Source: CAD feature listing. Evaluate the final solid. Frame: model axes, mm. A direction names the side the tool comes from. Give positions to 0.01 mm unless a question says otherwise; leave off trailing zeros. Loops run counter-clockwise (first coordinate to the right, second up) from the corner with the lowest first, then second, coordinate; pieces in that order, holes last. Notation, with made-up numbers: (29.25, 37) -> (38.25, 37) arc R18 ccw to (38.25, 54) -> close; hole circle Ø2 at (32.5, -11.5). An arc over 180 degrees is marked (long way). Return JSON: item names as keys, results as strings. Group by question number.
(1) Cut plane C-C on y = 28. Return loops of the section in (x, z).
(2) Access query for faces 4 (the face through (-35, 20, -22.5)), 5 (the face through (-1, 47, 32)), 6 (the face through (35, 20, -22.5)). Directions: +Z, -Z, +X, -X, +Y, -Y. A direction counts if a zero-diameter tool reaches every point of the face in a straight line with its end or side. Return the directions, or none.
(3) Ray query, line 1 (Z direction, x = 32.5, y = 18.5); line 2 (Y direction, x = -35.5, z = 12.5); line 3 (Z direction, x = 6.5, y = 15). Return the intervals inside material, ascending. Write a range as from..to.
(4) Cut plane D-D on x = -31.5. Return loops of the section in (y, z).
(5) Cut plane B-B on x = 0. Return loops of the section in (y, z).
(6) Cut plane A-A on z = 0. Return loops of the section in (x, y).
(7) Pin query (flat end, axial travel): pin 1 (6.5 mm diameter, centred on x = -7.5, y = 45.5, fed in from +Z); pin 2 (3 mm diameter, centred on x = 14, y = 47, fed in from -Z); pin 3 (6.5 mm diameter, centred on x = -5.5, z = -35.5, fed in from +Y); pin 4 (10 mm diameter, centred on y = 29, z = 0.5, fed in from +X). Return the tip coordinate at first contact, or that it passes through.
(8) Draft query along Z for faces 1 (the face through (37, 40, 0)), 2 (the face through (-1, 22, 38)), 3 (the face through (-1, 44, 35)). Return one class per face: released by +Z, released by -Z, zero draft, split by the parting line, or undercut.
```python
from build123d import *

# Parameters (mm, degrees)
CHANNEL_BODY_DEPTH      = 40
TOP_PLATE_SKETCH_W      = 100
TOP_PLATE_SKETCH_H      = 76
TOP_PLATE_DEPTH         = 10
BORE_SKETCH_R           = 12.5
BORE_25_DEPTH           = 56
GUIDE_GROOVES_SKETCH_W  = 100
GUIDE_GROOVES_SKETCH_H  = 6
GUIDE_GROOVES_6X6_DEPTH = 6


with BuildPart() as part:
    # Channel Profile Sketch → Channel Body (new body)
    with BuildSketch(Plane(origin=(0, 0, 0), x_dir=(1, 0, 0), z_dir=(0, 1, 0))):
        with BuildLine():
            Line((-50, 22.5), (-20.093531297, 22.5))
            ThreePointArc((-20.093531297, 22.5), (-17.330574806, 20.668790584), (-17.940652944, 17.410714286))
            ThreePointArc((-17.940652944, 17.410714286), (-25, 0), (-17.940652944, -17.410714286))
            ThreePointArc((-17.940652944, -17.410714286), (-17.330574806, -20.668790584), (-20.093531297, -22.5))
            Line((-20.093531297, -22.5), (-50, -22.5))
            Line((-50, -22.5), (-50, -38))
            Line((-50, -38), (50, -38))
            Line((50, -38), (50, -22.5))
            Line((50, -22.5), (20.093531297, -22.5))
            ThreePointArc((20.093531297, -22.5), (17.330574806, -20.668790584), (17.940652944, -17.410714286))
            ThreePointArc((17.940652944, -17.410714286), (25, 0), (17.940652944, 17.410714286))
            ThreePointArc((17.940652944, 17.410714286), (17.330574806, 20.668790584), (20.093531297, 22.5))
            Line((20.093531297, 22.5), (50, 22.5))
            Line((50, 22.5), (50, 38))
            Line((50, 38), (-50, 38))
            Line((-50, 38), (-50, 22.5))
        make_face()
    extrude(amount=CHANNEL_BODY_DEPTH)

    # Top Plate Sketch → Top Plate (add)
    with BuildSketch(Plane(origin=(0, 40, 0), x_dir=(1, 0, 0), z_dir=(0, 1, 0))):
        Rectangle(TOP_PLATE_SKETCH_W, TOP_PLATE_SKETCH_H)
    extrude(amount=TOP_PLATE_DEPTH)

    # Bore Sketch → Bore Ø25 (cut)
    with BuildSketch(Plane(origin=(0, 50, 0), x_dir=(1, 0, 0), z_dir=(0, 1, 0))):
        with Locations(Location((0, 0, 0), (0, 0, 270))):
            Circle(BORE_SKETCH_R)
    extrude(amount=-BORE_25_DEPTH, mode=Mode.SUBTRACT)

    # Guide Grooves Sketch → Guide Grooves 6x6 (cut)
    with BuildSketch(Plane(origin=(0, 50, 0), x_dir=(1, 0, 0), z_dir=(0, 1, 0))):
        with Locations((0, 35)):
            Rectangle(GUIDE_GROOVES_SKETCH_W, GUIDE_GROOVES_SKETCH_H)
        with Locations((0, -35)):
            Rectangle(GUIDE_GROOVES_SKETCH_W, GUIDE_GROOVES_SKETCH_H)
    extrude(amount=-GUIDE_GROOVES_6X6_DEPTH, mode=Mode.SUBTRACT)


solid = part.part
```
Answers:
{
 "1": {"outline": "(-50, -38) -> (50, -38) -> (50, -22.5) -> (20.09, -22.5) arc R3 cw to (17.94, -17.41) arc R25 ccw to (17.94, 17.41) arc R3 cw to (20.09, 22.5) -> (50, 22.5) -> (50, 38) -> (-50, 38) -> (-50, 22.5) -> (-20.09, 22.5) arc R3 cw to (-17.94, 17.41) arc R25 ccw to (-17.94, -17.41) arc R3 cw to (-20.09, -22.5) -> (-50, -22.5) -> close; hole circle Ø25 at (0, 0)"},
 "2": {"face 4": "-X, -Y", "face 5": "+Z, +X, -X, +Y", "face 6": "+X, -Y"},
 "3": {"line 1": "-38..-22.5, 22.5..38", "line 2": "40..50", "line 3": "-38..-10.68, 10.68..38"},
 "4": {"outline": "(0, -38) -> (44, -38) -> (44, -32) -> (50, -32) -> (50, 32) -> (44, 32) -> (44, 38) -> (0, 38) -> (0, 22.5) -> (40, 22.5) -> (40, -22.5) -> (0, -22.5) -> close"},
 "5": {"outline": "(0, -38) -> (44, -38) -> (44, -32) -> (50, -32) -> (50, -12.5) -> (0, -12.5) -> close; (0, 12.5) -> (50, 12.5) -> (50, 32) -> (44, 32) -> (44, 38) -> (0, 38) -> close"},
 "6": {"outline": "(-50, 40) -> (-25, 40) -> (-25, 0) -> (-12.5, 0) -> (-12.5, 50) -> (-50, 50) -> close; (12.5, 0) -> (25, 0) -> (25, 40) -> (50, 40) -> (50, 50) -> (12.5, 50) -> close"},
 "7": {"pin 1": "z = 38", "pin 2": "z = -32", "pin 3": "y = 44", "pin 4": "x = 25"},
 "8": {"face 1": "undercut", "face 2": "released by +Z", "face 3": "zero draft"}
}
